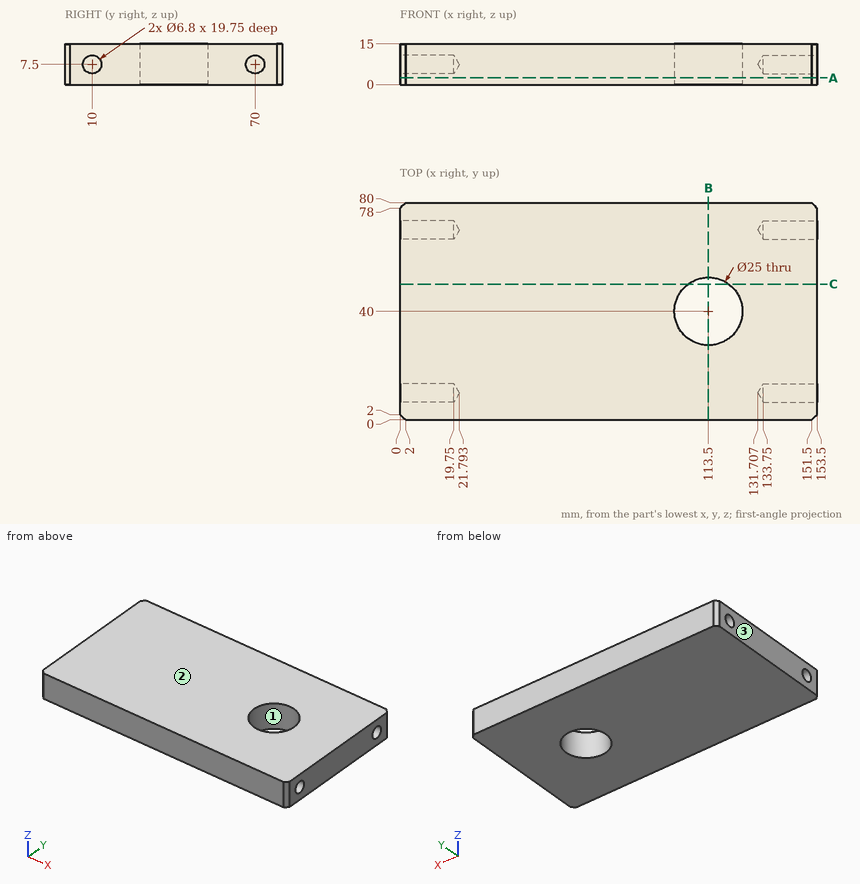
Can you work these out from the drawing? Everything is in mm from the part's minimum corner. Coordinates: 2 decimals unless noted, no trailing zeros. Loops run counter-clockwise (first coordinate to the right, second up) from the corner with the lowest first, then second, coordinate; pieces in that order, holes last. Notation, with made-up numbers: (-9, -15.5) - (22, -15.5) arc R9 ccw to (22, -1.5) - close; hole circle Ø10 at (22, 57). An arc over 180 degrees is marked (long way). Use a Markdown table: item, result.
Item 1: I want a section at B-B on x = 113.5. Please give me the cut outline in (y, z), and give its area (3 significant figures).
Numbers:
| item | result |
|---|---|
| outline | (0, 0) - (27.5, 0) - (27.5, 15) - (0, 15) - close; (52.5, 0) - (80, 0) - (80, 15) - (52.5, 15) - close |
| area | 825 mm2 |
Item 2: I want a section at C-C on y = 50. Please give me the cut outline in (x, z), and give its area (3 significant figures).
Numbers:
| item | result |
|---|---|
| outline | (0, 0) - (106, 0) - (106, 15) - (0, 15) - close; (121, 0) - (153.5, 0) - (153.5, 15) - (121, 15) - close |
| area | 2,080 mm2 |
Item 3: If I drill on probe 1 along Y at (x, z) = (138.25, 7.5); probe 2 along Z at (x, y) = (146.75, 70); probe 3 along Y at (x, z) = (113.5, 5.5), over which ranges is the centre line in solid material (lowest first)? Write a range as from..to.
Numbers:
| item | result |
|---|---|
| probe 1 | y = 0..6.6, 13.4..66.6, 73.4..80 |
| probe 2 | z = 0..4.1, 10.9..15 |
| probe 3 | y = 0..27.5, 52.5..80 |
Item 4: We'd pull the mould along X, two halves only. Please class the marked faces 1, 2 and 3: released by +X, released by -X, zero draft, split by the parting line, or undercut.
Numbers:
| item | result |
|---|---|
| face 1 | undercut |
| face 2 | zero draft |
| face 3 | released by -X |
Item 5: I want a section at A-A on z = 2.5. Please give me the cut outline in (x, y).
Numbers:
| item | result |
|---|---|
| outline | (0, 2) - (2, 0) - (151.5, 0) - (153.5, 2) - (153.5, 78) - (151.5, 80) - (2, 80) - (0, 78) - close; hole circle Ø25 at (113.5, 40) |
Item 6: Will these pins go through, and if not, where does the flat tip stop? pin 1 (4 mm diameter, centred on y = 70, z = 7.5, fed in from +X); pin 2 (20 mm diameter, centred on x = 113.5, y = 40, fed in from -Z); pin 3 (5.5 mm diameter, centred on y = 10, z = 7.5, fed in from +X); pin 4 (4 mm diameter, centred on y = 70, z = 7.5, fed in from -X).
Numbers:
| item | result |
|---|---|
| pin 1 | stops at x = 132.91 |
| pin 2 | passes through |
| pin 3 | stops at x = 133.36 |
| pin 4 | stops at x = 20.59 |
